```python
from build123d import *

# Parameters (mm, degrees)
SUPPORT_BLOCK_84MM_DEPTH = 84
TOP_BEVEL_CUT_DEPTH      = 84
SLOT_8MM_SKETCH_W        = 29.5
SLOT_8MM_SKETCH_H        = 8
SLOT_8MM_CUT_DEPTH       = 104
SLOT_8X21_CUT_DEPTH      = 104


with BuildPart() as part:
    # Block Profile Sketch → Support Block 84mm (new body)
    with BuildSketch(Plane(origin=(0, 0, 0), x_dir=(0, 0, -1), z_dir=(1, 0, 0))):
        Polygon((-23, 47), (-23, 10), (-35, 10), (-35, 0), (0, 0), (0, 71), (-20, 71), (-35, 60.496886927), (-35, 47), align=None)
    extrude(amount=-SUPPORT_BLOCK_84MM_DEPTH)

    # Top Bevel Sketch → Top Bevel Cut (cut)
    with BuildSketch(Plane.XY.offset(35)):
        Polygon((0, 35), (-11.689336678, 53), (-33.917485495, 71), (24.610458678, 71), (24.610458678, 35), align=None)
        Polygon((-50.082514505, 71), (-95.876326583, 71), (-95.876326583, 33.772958176), (-84, 35), (-72.310663322, 53), align=None)
    extrude(amount=-TOP_BEVEL_CUT_DEPTH, mode=Mode.SUBTRACT)

    # Slot 8mm Sketch → Slot 8mm Cut (cut)
    with BuildSketch(Plane(origin=(0, 71, 0), x_dir=(1, 0, 0), z_dir=(0, 1, 0))):
        with Locations((-69.25, -4)):
            Rectangle(SLOT_8MM_SKETCH_W, SLOT_8MM_SKETCH_H)
        with Locations((-14.75, -4)):
            Rectangle(SLOT_8MM_SKETCH_W, SLOT_8MM_SKETCH_H)
    extrude(amount=-SLOT_8MM_CUT_DEPTH, mode=Mode.SUBTRACT)

    # Slot 8x21 Sketch → Slot 8x21 Cut (cut)
    with BuildSketch(Plane.XY.offset(23)):
        with BuildLine():
            Line((-46, 18), (-46, 39))
            ThreePointArc((-46, 39), (-42, 43), (-38, 39))
            Line((-38, 39), (-38, 18))
            ThreePointArc((-38, 18), (-42, 14), (-46, 18))
        make_face()
    extrude(amount=-SLOT_8X21_CUT_DEPTH, mode=Mode.SUBTRACT)


solid = part.part
```
Geometry: final body of the model. Coordinates: model frame, mm. A direction names the side the tool comes from. Coordinates: 2 decimals unless noted, no trailing zeros. Order: outer loops, then holes, each group sorted by start corner. A loop starts at its lowest first (then second) coordinate and runs counter-clockwise, first axis right, second up. Notation, with made-up numbers: (-27.5, 77) - (-3.5, 77) arc R26 cw to (-3.5, 95) - close; hole circle Ø8 at (73.25, 13.5). An arc over 180 degrees is marked (long way). Return JSON: item names as keys, results as strings. Group by question number.
1. Set-up query: faces 1 (the face through (-29.5, 34, 4)), 2 (the face through (-69, 27, 8)), 3 (the face through (-41, 10, 29)), 4 (the face through (-42, 14, 12)). Return all of +Z, -Z, +X, -X, +Y, -Y with unobstructed straight access to the full face (end or side cutting, diameter ignored); none if empty.
2. Pin query (flat end, axial travel): pin 1 (1 mm diameter, centred on x = -31, z = 23, fed in from +Y); pin 2 (9.5 mm diameter, centred on x = -32, z = 31.5, fed in from +Y); pin 3 (10 mm diameter, centred on y = 61.5, z = 16, fed in from -X); pin 4 (3.5 mm diameter, centred on x = -29, z = 29, fed in from -Y). Return the tip coordinate at first contact, or that it passes through.
3. Cut plane C-C (y = 42). Output: boundary loops of the cut face in (x, z).
4. Cut plane B-B (z = 15). Output: boundary loops of the cut face in (x, y).
5. Material intervals for line 1 along X through (y, z) = (24, 14); line 2 along X through (y, z) = (38, 6.5); line 3 along X through (y, z) = (53, 6), sorted ascending. Write a range as [from, to].
6. Cut plane D-D (z = 27.5). Output: boundary loops of the cut face in (x, y).
7. Pull-direction query (X, two-part tool) for faces 5 (the face through (-42, 43, 12)), 6 (the face through (-22.648, 61.874, 17.745)), 7 (the face through (-41, 5, 35)); classes: pulls with the +X half, pulls with the -X half, needs draft (parallel to the pull), parting line crosses it, or undercut.
8. Cut plane A-A (x = -42). Output: boundary loops of the cut face in (y, z).
Resolved:
{
 "1": {"face 1": "-Z, +X, +Y, -Y", "face 2": "-Z, -X, +Y, -Y", "face 3": "+Z, +X, -X", "face 4": "+Z, -Z"},
 "2": {"pin 1": "stops at y = 69.02", "pin 2": "stops at y = 66.27", "pin 3": "stops at x = -67.99", "pin 4": "stops at y = 0"},
 "3": {"outline": "(-79.45, 8) - (-54.5, 8) - (-54.5, 0) - (-44.65, 0) - (-44.65, 23) - (-79.45, 23) - close; (-39.35, 0) - (-29.5, 0) - (-29.5, 8) - (-4.55, 8) - (-4.55, 23) - (-39.35, 23) - close"},
 "4": {"outline": "(-84, 0) - (0, 0) - (0, 35) - (-11.69, 53) - (-33.92, 71) - (-50.08, 71) - (-72.31, 53) - (-84, 35) - close; hole (-46, 18) arc R4 ccw to (-38, 18) - (-38, 39) arc R4 ccw to (-46, 39) - close"},
 "5": {"line 1": "x = [-84, -46], [-38, 0]", "line 2": "x = [-54.5, -46], [-38, -29.5]", "line 3": "x = [-54.5, -29.5]"},
 "6": {"outline": "(-84, 0) - (0, 0) - (0, 10) - (-84, 10) - close; (-76.21, 47) - (-7.79, 47) - (-11.69, 53) - (-27.43, 65.75) - (-56.57, 65.75) - (-72.31, 53) - close"},
 "7": {"face 5": "undercut", "face 6": "pulls with the +X half", "face 7": "needs draft"},
 "8": {"outline": "(0, 0) - (14, 0) - (14, 23) - (10, 23) - (10, 35) - (0, 35) - close; (43, 0) - (71, 0) - (71, 20) - (60.5, 35) - (47, 35) - (47, 23) - (43, 23) - close"}
}
